Geometry check sheet. Reference: drawing and pictorial views, mm from the part's lowest x, y, z. A direction names the side the tool comes from. Round coordinates to 2 decimals unless told otherwise and drop trailing zeros. Loops run counter-clockwise (first coordinate to the right, second up) from the corner with the lowest first, then second, coordinate; pieces in that order, holes last. Notation, with made-up numbers: (66, 21) - (112, 21) arc R17 cw to (112, 34) - close; hole circle Ø2 at (1, 22.25). An arc over 180 degrees is marked (long way). Answer in a Markdown table with one row per item. Add a question column.
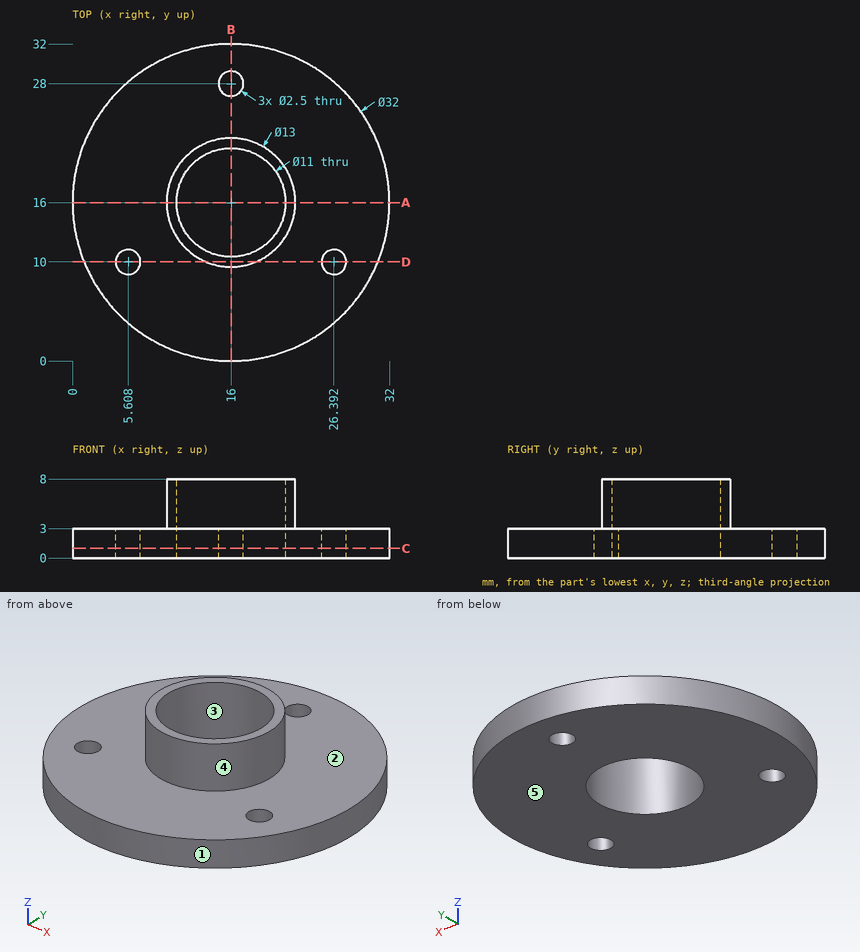
Q1. Set-up check for the marked faces 4 and 5: record each of +Z, -Z, +X, -X, +Y, -Y from which the full face is reachable in a straight line by a thin tool's end or side.
Q2. Cross-section at C-C, the plane z = 1. Enter the section's corners in (x, y).
Q3. Scan lines: line 1 (Y direction, x = 16, z = 1.4); line 2 (Y direction, x = 16, z = 4.25); line 3 (Z direction, x = 12.5, y = 23). Record each from-to range of solid material in increasing order. Write a range as from..to.
Q4. Cross-section at A-A, the plane y = 16. Enter the section's corners in (x, z).
Q5. Release check for a two-part mould opening along Y. For the marked faces 1, 2 and 3 record: +Y half, -Y half, draft (parallel to the pull), parting line (faces both ways), or undercut.
Q6. Cross-section at D-D, the plane y = 10. Enter the section's corners in (x, z).
Q7. Depth check by flat-ended pin: P1, Ø2, axis at x = 25.5, y = 28, coming from the +Z side; P2, Ø1.5, axis at y = 14.5, z = 5.5, coming from the -X side; P3, Ø1, axis at x = 7.5, z = 4, coming from the +Y side; P4, Ø1, axis at x = 8.5, z = 2, coming from the -Y side. Enter the tip coordinate at first touch or a pass-through.
Q8. Cross-section at B-B, the plane x = 16. Enter the section's corners in (y, z), plus the area to 3 significant figures.
Check sheet entries:
| question | item | result |
|---|---|---|
| 1 | face 4 | +Z |
| 1 | face 5 | -Z, +X, -X, +Y, -Y |
| 2 | outline | circle Ø32 at (16, 16); hole circle Ø2.5 at (5.61, 10); hole circle Ø11 at (16, 16); hole circle Ø2.5 at (16, 28); hole circle Ø2.5 at (26.39, 10) |
| 3 | line 1 | 0..10.5, 21.5..26.75, 29.25..32 |
| 3 | line 2 | 9.5..10.5, 21.5..22.5 |
| 3 | line 3 | 0..3 |
| 4 | outline | (0, 0) - (10.5, 0) - (10.5, 8) - (9.5, 8) - (9.5, 3) - (0, 3) - close; (21.5, 0) - (32, 0) - (32, 3) - (22.5, 3) - (22.5, 8) - (21.5, 8) - close |
| 5 | face 1 | parting line |
| 5 | face 2 | draft |
| 5 | face 3 | undercut |
| 6 | outline | (1.17, 0) - (4.36, 0) - (4.36, 3) - (1.17, 3) - close; (6.86, 0) - (25.14, 0) - (25.14, 3) - (18.5, 3) - (18.5, 8) - (13.5, 8) - (13.5, 3) - (6.86, 3) - close; (27.64, 0) - (30.83, 0) - (30.83, 3) - (27.64, 3) - close |
| 7 | P1 | z = 3 |
| 7 | P2 | x = 9.54 |
| 7 | P3 | through |
| 7 | P4 | y = 1.61 |
| 8 | outline | (0, 0) - (10.5, 0) - (10.5, 8) - (9.5, 8) - (9.5, 3) - (0, 3) - close; (21.5, 0) - (26.75, 0) - (26.75, 3) - (22.5, 3) - (22.5, 8) - (21.5, 8) - close; (29.25, 0) - (32, 0) - (32, 3) - (29.25, 3) - close |
| 8 | area | 65.5 mm² |
